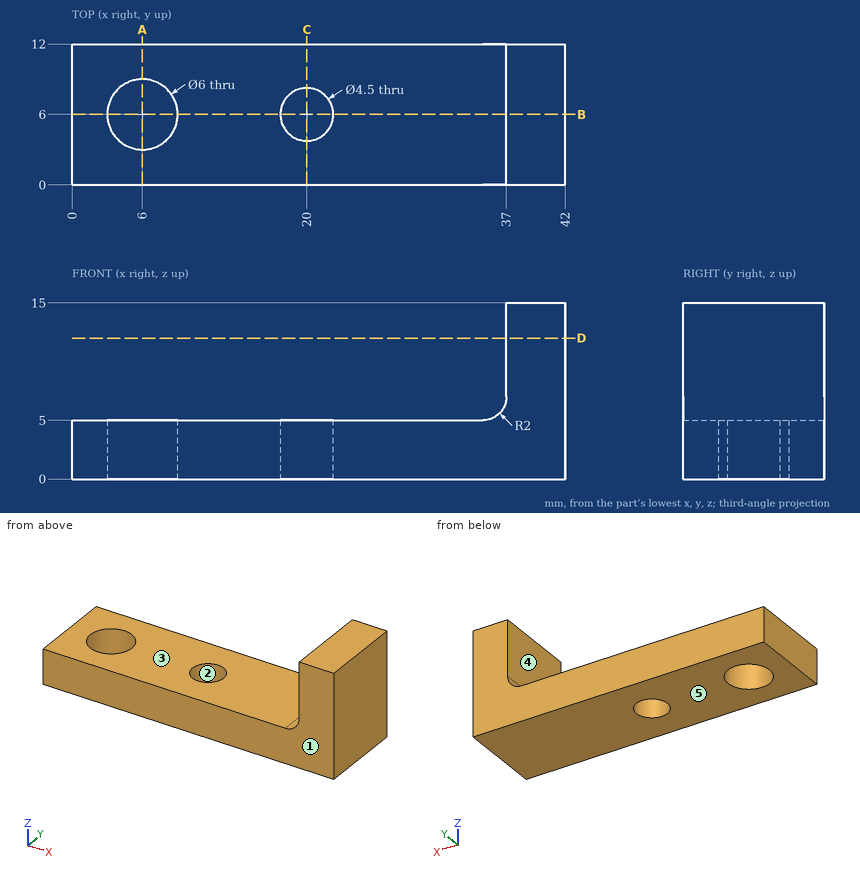
Study the drawing (mm; zero at the part's minimum x, y, z) and answer. A direction names the side the tool comes from. Give positions to 0.01 mm unless a question says otherwise; leave off trailing zeros. Order: outer loops, then holes, each group sorted by start corner. A loop starts at its lowest first (then second) coordinate and runs counter-clockwise, first axis right, second up. Notation, with made-up numbers: (78, 83) - (110, 83) arc R31 ccw to (110, 107) - close; hole circle Ø1 at (-38, 9.5). An arc over 180 degrees is marked (long way). Answer in a Markdown table with one row per item. Add a question column.
Q1. The part is cut by section D-D (z = 12). Determine the outline of the cut face in (x, y), then the cut area to 3 significant figures.
Q2. The part is cut by section C-C (x = 20). Determine the outline of the cut face in (y, z).
Q3. The part is cut by section A-A (x = 6). Determine the outline of the cut face in (y, z).
Q4. The part is cut by section B-B (y = 6). Determine the outline of the cut face in (x, z), then the cut area to 3 significant figures.
Q5. Find the intervals of material crossed by line 1 along Y through (x, z) = (20, 1.85); line 2 along X through (y, z) = (5.5, 2.25); line 3 along X through (y, z) = (7.5, 8), in increasing order. Write a range as [from, to].
Q6. For a pull along Y with two mould halves and no side action, classify the marked faces 1, 2 and 3 as released by +Y, released by -Y, zero draft, split by the parting line, or undercut.
Q7. Given P1, Ø1.5, axis at y = 7.5, z = 9.5, coming from the -X side; P2, Ø2, axis at x = 18, y = 8.5, coming from the +Z side, each flat-ended and moving along its own axis, determine where each tip first touches the part or whether it passes through.
Q8. Which of the six approach directions +Z, -Z, +X, -X, +Y, -Y give full straight-line access (tool end or side, diameter ignored) to the marked faces 4 and 5?
Determined:
| question | item | result |
|---|---|---|
| 1 | outline | (37, 0) - (42, 0) - (42, 12) - (37, 12) - close |
| 1 | area | 60.0 mm² |
| 2 | outline | (0, 0) - (3.75, 0) - (3.75, 5) - (0, 5) - close; (8.25, 0) - (12, 0) - (12, 5) - (8.25, 5) - close |
| 3 | outline | (0, 0) - (3, 0) - (3, 5) - (0, 5) - close; (9, 0) - (12, 0) - (12, 5) - (9, 5) - close |
| 4 | outline | (0, 0) - (3, 0) - (3, 5) - (0, 5) - close; (9, 0) - (17.75, 0) - (17.75, 5) - (9, 5) - close; (22.25, 0) - (42, 0) - (42, 15) - (37, 15) - (37, 7) arc R2 cw to (35, 5) - (22.25, 5) - close |
| 4 | area | 208 mm² |
| 5 | line 1 | y = [0, 3.75], [8.25, 12] |
| 5 | line 2 | x = [0, 3.04], [8.96, 17.81], [22.19, 42] |
| 5 | line 3 | x = [37, 42] |
| 6 | face 1 | released by -Y |
| 6 | face 2 | undercut |
| 6 | face 3 | zero draft |
| 7 | P1 | stops at x = 37 |
| 7 | P2 | stops at z = 5 |
| 8 | face 4 | +Z, -X, +Y, -Y |
| 8 | face 5 | -Z, +X, -X, +Y, -Y |
